Input: part model. Units: mm. Frame: model coordinates. A direction names the side the tool comes from. Coordinates: 2 decimals unless noted, no trailing zeros. Loops run counter-clockwise (first coordinate to the right, second up) from the corner with the lowest first, then second, coordinate; pieces in that order, holes last.
Item 1: Section B-B on x = 0. Return loops of the section in (y, z).
Item 2: Pull-direction query (Y, two-part tool) for faces 1 (the flat face through (0, 0, -0.5)), 2 (the flat face through (-2, -5, 0)), 3 (the flat face through (0, -0.75, -2)), 4 (the cylindrical face through (-1.08, -4.88, 34.26)); classes: released by +Y, released by -Y, zero draft, split by the parting line, or undercut.
Item 3: Reachability of faces 5 (the flat face through (0, 0.75, -2)), 6 (the flat face through (0, 0, 70)) from +Z, -Z, +X, -X, +Y, -Y: full face, straight path, thin tool, end or side. Return the list, or none.
Item 4: Contact query for flat-ended pins moving along their axis: P1, Ø0.8, axis at x = -3.5, y = 0, coming from the -Z side; P2, Ø6, axis at y = 1, z = 40, coming from the +X side; P3, Ø3, axis at y = -3, z = 38.5, coming from the -X side; P4, Ø5, axis at x = -4.5, y = 4, coming from the +Z side. Output: stop coordinate, or through.
Item 5: Section C-C on z = 39. Return loops of the section in (x, y).
Item 6: Section A-A on y = 0. Return loops of the section in (x, z).
Item 7: Ray query, line 1 along Z through (x, y) = (-4.5, -4.25); line 2 along Z through (x, y) = (6, -0.25); line 3 along Y through (x, z) = (-0.25, 7). Return the intervals inside material, ascending.
```python
from build123d import *

# Parameters (mm, degrees)
SKETCH_4_R          = 5
EXTRUDE_3_DEPTH     = 70
SKETCH_5_R          = 6.75
EXTRUDE_4_DEPTH     = 2.5
CHAMFER_1_SIZE      = 0.5
CHAMFER_2_SIZE      = 0.2
SKETCH_6_W          = 15
SKETCH_6_H          = 1.5
CUT_EXTRUDE_1_DEPTH = 2


with BuildPart() as part:
    # 草图4 → 凸台-拉伸3 (new body)
    with BuildSketch(Plane.XY):
        Circle(SKETCH_4_R)
    extrude(amount=EXTRUDE_3_DEPTH)

    # 草图5 → 凸台-拉伸4 (add)
    with BuildSketch(Plane(origin=(0, 0, 0), x_dir=(-1, 0, 0), z_dir=(0, 0, -1))):
        Circle(SKETCH_5_R)
    extrude(amount=EXTRUDE_4_DEPTH)

    # 倒角1
    chamfer_1_edges = [part.edges().sort_by_distance(p)[0] for p in [
        (-5, 0, 70),
    ]]
    chamfer(chamfer_1_edges, length=CHAMFER_1_SIZE)

    # 倒角2
    chamfer_2_edges = [part.edges().sort_by_distance(p)[0] for p in [
        (6.75, 0, 0),
        (6.75, 0, -2.5),
    ]]
    chamfer(chamfer_2_edges, length=CHAMFER_2_SIZE)

    # 草图6 → 切除-拉伸1 (cut)
    with BuildSketch(Plane(origin=(0, 0, -2.5), x_dir=(-1, 0, 0), z_dir=(0, 0, -1))):
        Rectangle(SKETCH_6_W, SKETCH_6_H)
    extrude(amount=-CUT_EXTRUDE_1_DEPTH, mode=Mode.SUBTRACT)


solid = part.part
```
Results found:
1. outline: (-6.75, -2.3) - (-6.55, -2.5) - (-0.75, -2.5) - (-0.75, -0.5) - (0.75, -0.5) - (0.75, -2.5) - (6.55, -2.5) - (6.75, -2.3) - (6.75, -0.2) - (6.55, 0) - (5, 0) - (5, 69.5) - (4.5, 70) - (-4.5, 70) - (-5, 69.5) - (-5, 0) - (-6.55, 0) - (-6.75, -0.2) - close
2. face 1: undercut
2. face 2: zero draft
2. face 3: undercut
2. face 4: split by the parting line
3. face 5: -Z, +X, -X
3. face 6: +Z, +X, -X, +Y, -Y
4. P1: stops at z = -0.5
4. P2: stops at x = 5
4. P3: stops at x = -4.77
4. P4: stops at z = 70
5. outline: circle Ø10 at (0, 0)
6. outline: (-6.75, -0.5) - (6.75, -0.5) - (6.75, -0.2) - (6.55, 0) - (5, 0) - (5, 69.5) - (4.5, 70) - (-4.5, 70) - (-5, 69.5) - (-5, 0) - (-6.55, 0) - (-6.75, -0.2) - close
7. line 1: z = -2.5 to 0
7. line 2: z = -0.5 to 0
7. line 3: y = -4.99 to 4.99
